from build123d import *

# Parameters (mm, degrees)
SKETCH1_W           = 130
SKETCH1_H           = 50
BOSS_EXTRUDE1_DEPTH = 10
SKETCH2_R           = 5
CUT_EXTRUDE1_DEPTH  = 2


with BuildPart() as part:
    # Sketch1 → Boss-Extrude1 (new body)
    with BuildSketch(Plane.XY):
        Rectangle(SKETCH1_W, SKETCH1_H)
    extrude(amount=BOSS_EXTRUDE1_DEPTH)

    # Sketch2 → Cut-Extrude1 (cut)
    with BuildSketch(Plane.XY.offset(10)):
        with Locations((-37.5, 0)):
            Circle(SKETCH2_R)
        with Locations((-22.5, 0)):
            Circle(SKETCH2_R)
        with Locations((-7.5, 0)):
            Circle(SKETCH2_R)
        with Locations((7.5, 0)):
            Circle(SKETCH2_R)
        with Locations((22.5, 0)):
            Circle(SKETCH2_R)
        with Locations((37.5, 0)):
            Circle(SKETCH2_R)
    extrude(amount=-CUT_EXTRUDE1_DEPTH, mode=Mode.SUBTRACT)


solid = part.part
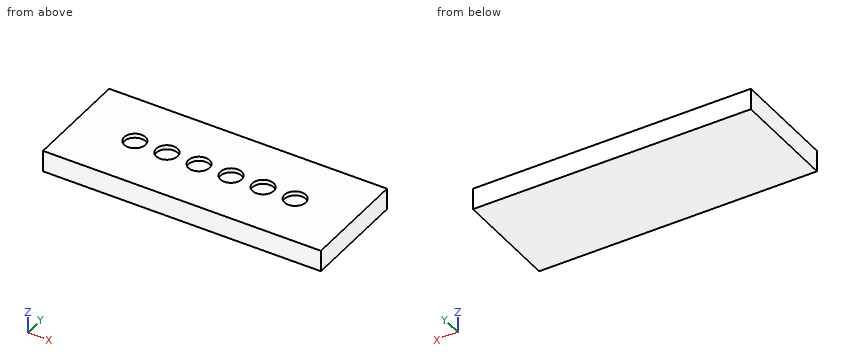
For this review, take the finished solid that the model builds, in its own axes (mm). Round coordinates to 2 decimals unless told otherwise and drop trailing zeros. Write each loop counter-clockwise with the first axis right and the second up, starting at its lowest first coordinate (ties: lowest second). Pieces come first, ordered by that corner, then holes. Notation, with made-up numbers: (5.25, 40.5) - (33.25, 40.5) arc R17 ccw to (33.25, 45.5) - close; hole circle Ø4 at (72.5, -32.75). An arc over 180 degrees is marked (long way). Write item = value, one per line. Start each with the question number.
1. Consider section C-C on x = 22.5. State the section outline as (y, z) points, plus the area to 3 significant figures.
2. For pin 1 Ø6 at (x, y) = (7.5, 0) entering from +Z, flat-tipped, find the tip position at first contact; note if it passes through.
3. Consider section B-B on y = 0. State the section outline as (x, z) points.
4. Consider section A-A on x = -4.5. State the section outline as (y, z) points.
5. Wall thickness on L1, parallel to Y at x = 22.5, z = 9.5; L2, parallel to Z at x = -41, y = -3; L3, parallel to Y at x = -33, z = 8.75: over which ranges is each line inside the solid? List them lowest first.
Evaluation:
q1.outline = (-25, 0) - (25, 0) - (25, 10) - (5, 10) - (5, 8) - (-5, 8) - (-5, 10) - (-25, 10) - close
q1.area = 480 mm2
q2.pin_1 = 8
q3.outline = (-65, 0) - (65, 0) - (65, 10) - (42.5, 10) - (42.5, 8) - (32.5, 8) - (32.5, 10) - (27.5, 10) - (27.5, 8) - (17.5, 8) - (17.5, 10) - (12.5, 10) - (12.5, 8) - (2.5, 8) - (2.5, 10) - (-2.5, 10) - (-2.5, 8) - (-12.5, 8) - (-12.5, 10) - (-17.5, 10) - (-17.5, 8) - (-27.5, 8) - (-27.5, 10) - (-32.5, 10) - (-32.5, 8) - (-42.5, 8) - (-42.5, 10) - (-65, 10) - close
q4.outline = (-25, 0) - (25, 0) - (25, 10) - (4, 10) - (4, 8) - (-4, 8) - (-4, 10) - (-25, 10) - close
q5.L1 = -25 to -5, 5 to 25
q5.L2 = 0 to 8
q5.L3 = -25 to -2.18, 2.18 to 25
